For this review, take the finished solid that the model builds, in its own axes (mm). A direction names the side the tool comes from. Coordinates: 2 decimals unless noted, no trailing zeros. Loops run counter-clockwise (first coordinate to the right, second up) from the corner with the lowest first, then second, coordinate; pieces in that order, holes last.
```python
from build123d import *

# Parameters (mm, degrees)
EXTRUDE_1_DEPTH        = 400
SHELL_1_T              = -2
SKETCH_3_W             = 650
SKETCH_3_H             = 600
CUT_EXTRUDE_1_DEPTH    = 2
SKETCH_4_W             = 654
SKETCH_4_H             = 604
SKETCH_4_W_2           = 650
SKETCH_4_H_2           = 600
EXTRUDE_2_DEPTH        = 24
SKETCH_5_W             = 654
SKETCH_5_H             = 604
SKETCH_5_W_2           = 614
SKETCH_5_H_2           = 564
EXTRUDE_3_DEPTH        = 2
EXTRUDE_4_DEPTH        = 2
CUT_EXTRUDE_2_DEPTH    = 2
SKETCH_10_W            = 666
SKETCH_10_H            = 2
EXTRUDE_7_DEPTH        = 28
SKETCH_12_R            = 4.5
CUT_EXTRUDE_3_DEPTH    = 10
SKETCH_13_R            = 4.5
CUT_EXTRUDE_4_DEPTH    = 10
SKETCH_14_R            = 4.5
CUT_EXTRUDE_5_DEPTH    = 10
HOLE_WIZARD_M5_1_D     = 4.2
HOLE_WIZARD_M5_1_DEPTH = 3
HOLE_WIZARD_M5_1_TIP   = 1.2618073


with BuildPart() as part:
    # 草图1 → 凸台-拉伸1 (new body)
    with BuildSketch(Plane(origin=(0, 0, 0), x_dir=(1, 0, 0), z_dir=(0, 1, 0))):
        Polygon((-425, 380), (-425, -290), (-325, -390), (425, -390), (425, 380), align=None)
    extrude(amount=-EXTRUDE_1_DEPTH)

    # 抽壳1
    shell_1_openings = [part.faces().sort_by_distance(p)[0] for p in [
        (3.015139851, -400, 2.292789325),
    ]]
    offset(amount=SHELL_1_T, openings=shell_1_openings, kind=Kind.INTERSECTION)

    # 草图3 → 切除-拉伸1 (cut)
    with BuildSketch(Plane(origin=(0, 0, 0), x_dir=(1, 0, 0), z_dir=(0, 1, 0))):
        Rectangle(SKETCH_3_W, SKETCH_3_H)
    extrude(amount=-CUT_EXTRUDE_1_DEPTH, mode=Mode.SUBTRACT)

    # 草图4 → 凸台-拉伸2 (add)
    with BuildSketch(Plane(origin=(0, 0, 0), x_dir=(1, 0, 0), z_dir=(0, 1, 0))):
        Rectangle(SKETCH_4_W, SKETCH_4_H)
        Rectangle(SKETCH_4_W_2, SKETCH_4_H_2, mode=Mode.SUBTRACT)
    extrude(amount=-EXTRUDE_2_DEPTH)

    # 草图5 → 凸台-拉伸3 (add)
    with BuildSketch(Plane.XZ.offset(24)):
        Rectangle(SKETCH_5_W, SKETCH_5_H)
        Rectangle(SKETCH_5_W_2, SKETCH_5_H_2, mode=Mode.SUBTRACT)
    extrude(amount=-EXTRUDE_3_DEPTH)

    # 草图6 → 凸台-拉伸4 (add)
    with BuildSketch(Plane.XZ.offset(400)):
        Polygon((-425, 290), (-325, 390), (425, 390), (425, 360), (-312.573593129, 360), (-403.786796564, 268.786796564), align=None)
    extrude(amount=-EXTRUDE_4_DEPTH)

    # 草图7 → 切除-拉伸2 (cut)
    with BuildSketch(Plane(origin=(425, 0, 0), x_dir=(0, 0, -1), z_dir=(1, 0, 0))):
        with BuildLine():
            Line((-310, -400), (-310, -305))
            ThreePointArc((-310, -305), (-270, -265), (-230, -305))
            Line((-230, -305), (-230, -400))
            Line((-230, -400), (-310, -400))
        make_face()
    extrude(amount=-CUT_EXTRUDE_2_DEPTH, mode=Mode.SUBTRACT)

    # 草图10 → 凸台-拉伸7 (add)
    with BuildSketch(Plane(origin=(-423, 0, 0), x_dir=(0, 0, -1), z_dir=(1, 0, 0))):
        with Locations((45, -399)):
            Rectangle(SKETCH_10_W, SKETCH_10_H)
    extrude(amount=EXTRUDE_7_DEPTH)

    # 草图12 → 切除-拉伸3 (cut)
    with BuildSketch(Plane(origin=(0, -398, 0), x_dir=(1, 0, 0), z_dir=(0, 1, 0))):
        with Locations(Location((-409, 350, 0), (0, 0, 270))):
            Circle(SKETCH_12_R)
        with Locations(Location((-363.686291501, -328.686291501, 0), (0, 0, 270))):
            Circle(SKETCH_12_R)
        with Locations(Location((-85, -374, 0), (0, 0, 270))):
            Circle(SKETCH_12_R)
        with Locations(Location((395, -374, 0), (0, 0, 270))):
            Circle(SKETCH_12_R)
        with Locations(Location((-409, -90, 0), (0, 0, 270))):
            Circle(SKETCH_12_R)
        with Locations(Location((-25, -374, 0), (0, 0, 270))):
            Circle(SKETCH_12_R)
        with Locations(Location((-409, -150, 0), (0, 0, 270))):
            Circle(SKETCH_12_R)
        with Locations(Location((23, -374, 0), (0, 0, 270))):
            Circle(SKETCH_12_R)
        with Locations(Location((123, -374, 0), (0, 0, 270))):
            Circle(SKETCH_12_R)
    extrude(amount=-CUT_EXTRUDE_3_DEPTH, mode=Mode.SUBTRACT)

    # 草图13 → 切除-拉伸4 (cut)
    with BuildSketch(Plane.XY.offset(-378)):
        with Locations((0, -30)):
            Circle(SKETCH_13_R)
        with Locations((-295, -30)):
            Circle(SKETCH_13_R)
        with Locations((0, -370)):
            Circle(SKETCH_13_R)
        with Locations((-295, -370)):
            Circle(SKETCH_13_R)
        with Locations((-395, -30)):
            Circle(SKETCH_13_R)
        with Locations((-395, -370)):
            Circle(SKETCH_13_R)
        with Locations(Location((295, -30, 0), (0, 0, 180))):
            Circle(SKETCH_13_R)
        with Locations(Location((295, -370, 0), (0, 0, 180))):
            Circle(SKETCH_13_R)
        with Locations(Location((395, -370, 0), (0, 0, 180))):
            Circle(SKETCH_13_R)
        with Locations(Location((395, -30, 0), (0, 0, 180))):
            Circle(SKETCH_13_R)
    extrude(amount=-CUT_EXTRUDE_4_DEPTH, mode=Mode.SUBTRACT)

    # 草图14 → 切除-拉伸5 (cut)
    with BuildSketch(Plane(origin=(425, 0, 0), x_dir=(0, 0, -1), z_dir=(1, 0, 0))):
        with Locations((-360, -230)):
            Circle(SKETCH_14_R)
        with Locations((-360, -370)):
            Circle(SKETCH_14_R)
        with Locations((-5, -230)):
            Circle(SKETCH_14_R)
        with Locations((-5, -370)):
            Circle(SKETCH_14_R)
        with Locations((350, -370)):
            Circle(SKETCH_14_R)
        with Locations((350, -230)):
            Circle(SKETCH_14_R)
    extrude(amount=-CUT_EXTRUDE_5_DEPTH, mode=Mode.SUBTRACT)

    # M5 螺纹孔1
    with Locations(Plane(origin=(425, 0, 0), x_dir=(0, 0, -1), z_dir=(1, 0, 0))):
        with Locations((-243, -258.234628196), (-216, -305), (-315, -359)):
            Hole(HOLE_WIZARD_M5_1_D / 2, depth=HOLE_WIZARD_M5_1_DEPTH)
            with Locations((0, 0, -(HOLE_WIZARD_M5_1_DEPTH + HOLE_WIZARD_M5_1_TIP / 2))):  # 118° drill point
                Cone(0, HOLE_WIZARD_M5_1_D / 2, HOLE_WIZARD_M5_1_TIP, mode=Mode.SUBTRACT)


solid = part.part
```
Q1. Machinability: for faces 5 (the face through (6, -197, -380)), 6 (the face through (-327, -13, 4)), 7 (the face through (-425, -197, -50)), 8 (the face through (-5, -11, -300)), 9 (the face through (-190, -398, 376)), which of the approach directions +Z, -Z, +X, -X, +Y, -Y give a long, thin tool a straight path to every point of the face, cutting with its end or side? Answer none if there is none.
Q2. Consider section A-A (x = -196.5). State the section outline as (y, z) points.
Q3. Consider section B-B (y = -126). State the section outline as (x, z) points.
Q4. For pin 1 Ø11.5 at (x, z) = (-363.69, 328.69) entering from +Y; pin 2 Ø5.5 at (x, y) = (0, -370) entering from -Z, all flat-tipped, find the tip position at first contact; note any pin that passes through.
Q5. Wall thickness on probe 1 along X at (y, z) = (-370, -379.45); probe 2 along X at (y, z) = (-399, 90); probe 3 along Y at (x, z) = (0, -379.25): over which ranges is each line inside the solid? List them lowest first.
Q6. The part is to be moulded in two halves that separate along X. For faces 1 (the face through (6, -198, -378)), 2 (the face through (45, -197, 390)), 3 (the face through (-376, -197, 339)), 4 (the face through (425, -197, 10)), say which applies: +X half, -X half, draft (parallel to the pull), parting line (faces both ways), or undercut.
Model answer:
1. face 5: -Z, +X, -X, +Y, -Y
1. face 6: -Y
1. face 7: +Z, -Z, -X, +Y, -Y
1. face 8: +Y
1. face 9: none
2. outline: (-400, -380) - (0, -380) - (0, -300) - (-22, -300) - (-22, -282) - (-24, -282) - (-24, -302) - (-2, -302) - (-2, -378) - (-400, -378) - close; (-400, 360) - (-398, 360) - (-398, 388) - (-2, 388) - (-2, 302) - (-24, 302) - (-24, 282) - (-22, 282) - (-22, 300) - (0, 300) - (0, 390) - (-400, 390) - close
3. outline: (-425, -380) - (425, -380) - (425, 390) - (-325, 390) - (-425, 290) - close; hole (-423, -378) - (423, -378) - (423, 388) - (-324.17, 388) - (-423, 289.17) - close
4. pin 1: stops at y = 0
4. pin 2: stops at z = 388
5. probe 1: x = -425 to -399.5, -390.5 to -299.5, -290.5 to -4.5, 4.5 to 290.5, 299.5 to 390.5, 399.5 to 425
5. probe 2: x = -425 to -413.5, -404.5 to -395, 423 to 425
5. probe 3: y = -400 to -374.5, -365.5 to -34.5, -25.5 to 0
6. face 1: undercut
6. face 2: draft
6. face 3: -X half
6. face 4: +X half
